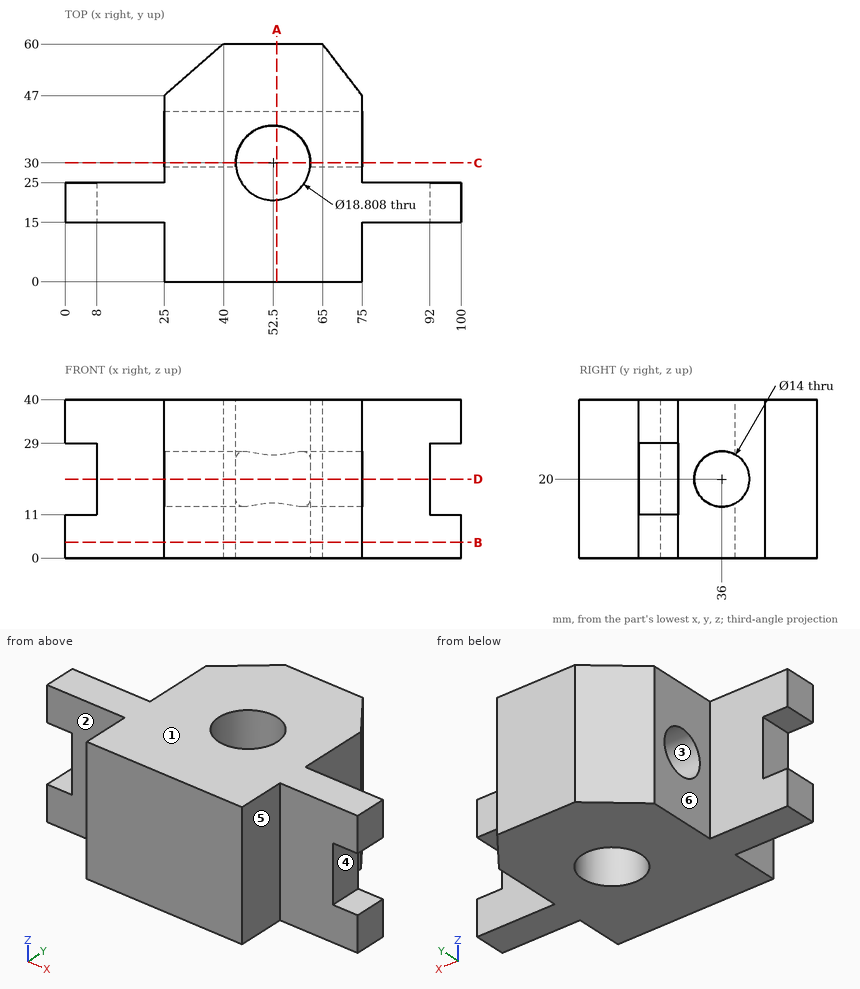
Check sheet for the drawn part. Datum: minimum x, y, z corner. Units: mm. A direction names the side the tool comes from. Coordinates: 2 decimals unless noted, no trailing zeros. Write each loop counter-clockwise with the first axis right and the second up, starting at its lowest first coordinate (ties: lowest second). Pieces come first, ordered by that corner, then holes. Notation, with made-up numbers: M 72.25,-30.75 L 123.25,-30.75 A24 ccw 123.25,-8.75 Z; hole C -13.5,29 d9. An arc over 180 degrees is marked long. Use a Markdown table: item, result.
Q1. Thickness scan on line 1 (Z direction, x = 39, y = 36); line 2 (Y direction, x = 52.5, z = 12); line 3 (X direction, y = 30, z = 9.5). Record the ranges inside material, lowest first.
Reply:
| item | result |
|---|---|
| line 1 | z = 0 to 13, 27 to 40 |
| line 2 | y = 0 to 20.6, 39.4 to 60 |
| line 3 | x = 25 to 43.1, 61.9 to 75 |
Q2. Sectioned sample at B-B, the plane z = 4. Record the boundary of the cut face in (x, y), plus the area to 3 significant figures.
Reply:
| item | result |
|---|---|
| outline | M 0,15 L 25,15 L 25,0 L 75,0 L 75,15 L 100,15 L 100,25 L 75,25 L 75,47 L 65,60 L 40,60 L 25,47 L 25,25 L 0,25 Z; hole C 52.5,30 d18.81 |
| area | 3,060 mm² |
Q3. Go/stop test with flat-tipped pins: P1, Ø20, axis at x = 6.5, z = 12, coming from the +Y side; P2, Ø10, axis at y = 48, z = 8, coming from the +X side; P3, Ø3, axis at x = 67.5, z = 4.5, coming from the +Y side; P4, Ø17, axis at x = 52.5, y = 30, coming from the +Z side. Record where each tip stops, or that it passes through.
Reply:
| item | result |
|---|---|
| P1 | stops at y = 25 |
| P2 | stops at x = 75 |
| P3 | stops at y = 58.7 |
| P4 | passes through |
Q4. Sectioned sample at D-D, the plane z = 20. Record the boundary of the cut face in (x, y), plus the area to 3 significant figures.
Reply:
| item | result |
|---|---|
| outline | M 8,15 L 25,15 L 25,0 L 75,0 L 75,15 L 92,15 L 92,25 L 75,25 L 75,29 L 61.85,29 A9.4 cw 43.15,29 L 25,29 L 25,25 L 8,25 Z; M 25,43 L 75,43 L 75,47 L 65,60 L 40,60 L 25,47 Z |
| area | 2,360 mm² |
Q5. Sectioned sample at A-A, the plane x = 53.5. Record the boundary of the cut face in (y, z).
Reply:
| item | result |
|---|---|
| outline | M 0,0 L 20.65,0 L 20.65,40 L 0,40 Z; M 39.35,0 L 60,0 L 60,40 L 39.35,40 L 39.35,26.15 A7 cw 39.35,13.85 Z |
Q6. Draft check along Z on the marked faces 1, 2 and 3. Enter one of: +Z half, -Z half, draft (parallel to the pull), parting line (faces both ways), or undercut.
Reply:
| item | result |
|---|---|
| face 1 | +Z half |
| face 2 | draft |
| face 3 | undercut |
Q7. Set-up check for the marked faces 4, 5 and 6: record each of +Z, -Z, +X, -X, +Y, -Y from which the full face is reachable in a straight line by a thin tool's end or side.
Reply:
| item | result |
|---|---|
| face 4 | +X, +Y, -Y |
| face 5 | +Z, -Z, +X, -Y |
| face 6 | +Z, -Z, -X, +Y |
Q8. Sectioned sample at C-C, the plane y = 30. Record the boundary of the cut face in (x, z) (1 decimal), plus the area to 3 significant figures.
Reply:
| item | result |
|---|---|
| outline | M 25,0 L 43.1,0 L 43.1,16.4 L 25,16.4 Z; M 25,23.6 L 43.1,23.6 L 43.1,40 L 25,40 Z; M 61.9,0 L 75,0 L 75,16.4 L 61.9,16.4 Z; M 61.9,23.6 L 75,23.6 L 75,40 L 61.9,40 Z |
| area | 1,020 mm² |
